Design review of the part built by this model. Coordinates are the model's own, in mm. A direction names the side the tool comes from. Coordinates: 2 decimals unless noted, no trailing zeros. Write each loop counter-clockwise with the first axis right and the second up, starting at its lowest first coordinate (ties: lowest second). Pieces come first, ordered by that corner, then holes. Notation, with made-up numbers: (48.5, 29.25) - (78.5, 29.25) arc R13 ccw to (78.5, 40.25) - close; hole circle Ø7 at (-6, 15). An arc over 180 degrees is marked (long way). One line per item, written item: value.
from build123d import *

# Parameters (mm, degrees)
BASE_PLATE_DEPTH        = 10
TAPERED_BOSS_DEPTH      = 70
TOP_SLOT_PROFILE_W      = 92.427210419
TOP_SLOT_PROFILE_H      = 20
TOP_SLOT_PROFILE_W_2    = 89.987361697
TOP_SLOT_CUT_19MM_DEPTH = 19


with BuildPart() as part:
    # Base Plate Profile → Base Plate (new body)
    with BuildSketch(Plane.XY):
        Polygon((-45, -15), (-45, -35), (45, -35), (45, -15), (40, -15), (40, 15), (45, 15), (45, 35), (-45, 35), (-45, 15), (-40, 15), (-40, -15), align=None)
    extrude(amount=BASE_PLATE_DEPTH)

    # Tapered Boss Profile → Tapered Boss (add)
    with BuildSketch(Plane(origin=(0, 35, 0), x_dir=(1, 0, 0), z_dir=(0, 1, 0))):
        Polygon((-25.475364852, 49), (-35, 0), (35, 0), (25.475364852, 49), align=None)
    extrude(amount=-TAPERED_BOSS_DEPTH)

    # Top Slot Profile → Top Slot Cut 19mm (cut)
    with BuildSketch(Plane(origin=(0, 0, -49), x_dir=(-1, 0, 0), z_dir=(0, 0, -1))):
        with Locations((7.299783504, 25)):
            Rectangle(TOP_SLOT_PROFILE_W, TOP_SLOT_PROFILE_H)
        with Locations((6.079859143, -25)):
            Rectangle(TOP_SLOT_PROFILE_W_2, TOP_SLOT_PROFILE_H)
    extrude(amount=-TOP_SLOT_CUT_19MM_DEPTH, mode=Mode.SUBTRACT)


solid = part.part
1. Consider section B-B, the plane x = 7.5. Write out the cut boundary in (y, z), then the cut area to 3 significant figures.
Answer block:
outline: (-35, -30) - (-15, -30) - (-15, -49) - (15, -49) - (15, -30) - (35, -30) - (35, 10) - (-35, 10) - close
area: 3,370 mm^2
2. Mouldability with a two-part tool opening along Y and no side actions: class faces 5 (the face through (0, -15, -40)), 6 (the face through (-40, 0, 5)), 7 (the face through (0, 25, -30)) as released by +Y, released by -Y, zero draft, split by the parting line, or undercut.
Answer block:
face 5: released by -Y
face 6: undercut
face 7: zero draft
3. Insertion check: pin 1 Ø5.5 at (x, z) = (-13, -38) entering from -Y; pin 2 Ø10 at (x, y) = (7.5, 21) entering from -Z; pin 3 Ø5 at (x, y) = (-39.5, -5) entering from -Z. Each pin has a flat end and moves straight along its axis. Give the tip position at first contact, or say it passes through.
Answer block:
pin 1: stops at y = -15
pin 2: stops at z = -30
pin 3: stops at z = 0
4. Consider section D-D, the plane x = -36.5. Write out the cut boundary in (y, z).
Answer block:
outline: (-35, 0) - (35, 0) - (35, 10) - (-35, 10) - close
5. Consider section A-A, the plane y = 4. Write out the cut boundary in (x, z).
Answer block:
outline: (-40, 0) - (-35, 0) - (-25.48, -49) - (25.48, -49) - (35, 0) - (40, 0) - (40, 10) - (-40, 10) - close
6. Consider section C-C, the plane z = -43.5. Write out the cut boundary in (x, y), then the cut area to 3 significant figures.
Answer block:
outline: (-26.54, -15) - (26.54, -15) - (26.54, 15) - (-26.54, 15) - close
area: 1,590 mm^2
7. Wall thickness on line 1 along Y through (x, z) = (-5, -40.5); line 2 along X through (y, z) = (1.5, 2); line 3 along Z through (x, y) = (23, 24): over which ranges is each line inside the solid? List them lowest first.
Answer block:
line 1: y = -15 to 15
line 2: x = -40 to 40
line 3: z = -30 to 10
8. For faces 1 (the face through (0, -25, -30)), 2 (the face through (-39, 0, 0)), 3 (the face through (43, -15, 5)), 4 (the face through (0, 15, -40)), list the 3-axis set-ups (+Z, -Z, +X, -X, +Y, -Y) from which the entire face can be reached by the end or side of a thin tool; tool diameter is ignored.
Answer block:
face 1: -Z, +X, -X, -Y
face 2: -Z, -X, +Y, -Y
face 3: +Z, -Z, +X
face 4: -Z, +X, -X, +Y
